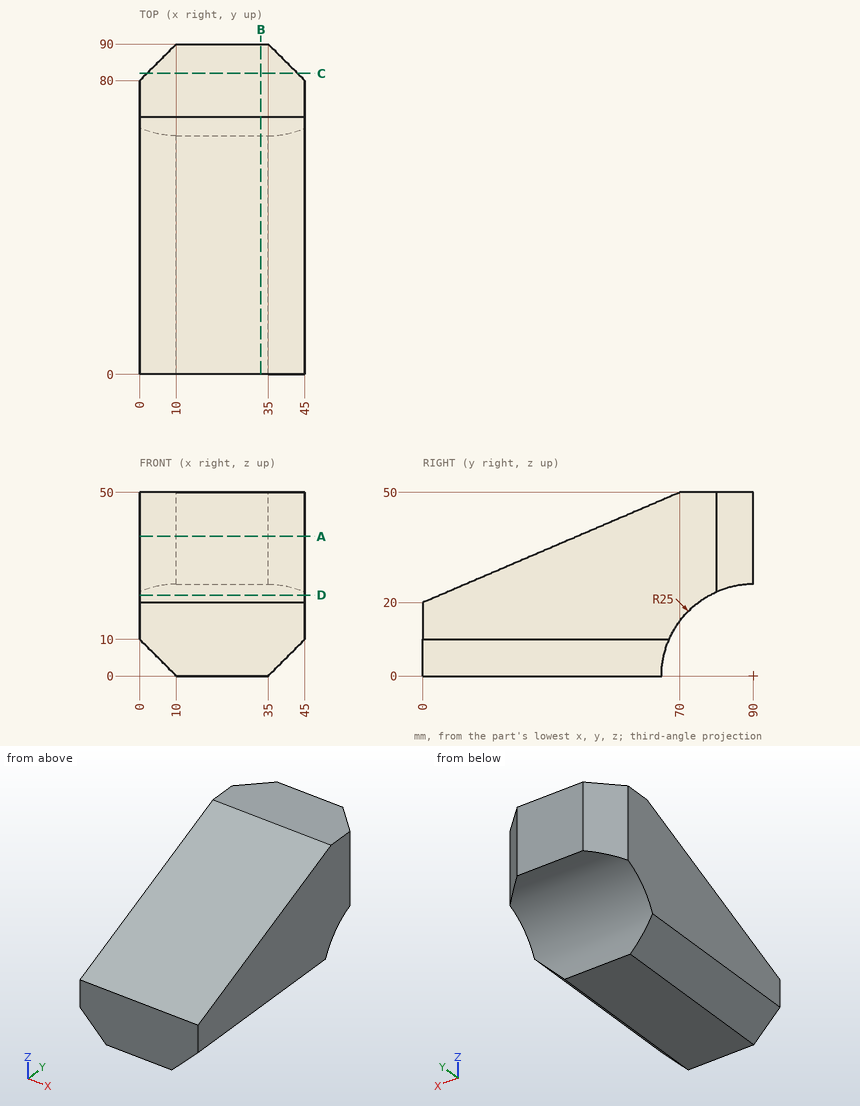
Geometry check sheet. Reference: drawing and pictorial views, mm from the part's lowest x, y, z. Give positions to 0.01 mm unless a question says otherwise; leave off trailing zeros. Loops run counter-clockwise (first coordinate to the right, second up) from the corner with the lowest first, then second, coordinate; pieces in that order, holes last.
1. Section check C-C, the plane y = 82. Enter the section's corners in (x, z), then the cut area to 3 significant figures.
2. Section check D-D, the plane z = 22. Enter the section's corners in (x, y), then the cut area to 3 significant figures.
3. Section check A-A, the plane z = 38. Enter the section's corners in (x, y).
4. Thickness scan on line 1 (Z direction, x = 35, y = 80); line 2 (Z direction, x = 27, y = 54); line 3 (Y direction, x = 25, z = 41.5). Record the ranges inside material, lowest first.
5. Go/stop test with flat-tipped pins: pin 1 Ø12 at (x, z) = (8.5, 33.5) entering from +Y; pin 2 Ø3 at (x, z) = (31, 8.5) entering from +Y; pin 3 Ø5 at (x, z) = (40, 27.5) entering from +Y; pin 4 Ø8 at (x, y) = (21.5, 29) entering from +Z. Record where each tip stops, or that it passes through.
6. Section check B-B, the plane x = 33. Enter the section's corners in (y, z), then the cut area to 3 significant figures.
Geometry says:
1. outline: (2, 23.69) - (43, 23.69) - (43, 50) - (2, 50) - close
1. area: 1,080 mm2
2. outline: (0, 4.67) - (45, 4.67) - (45, 78.13) - (0, 78.13) - close
2. area: 3,310 mm2
3. outline: (0, 42) - (45, 42) - (45, 80) - (35, 90) - (10, 90) - (0, 80) - close
4. line 1: z = 22.91 to 50
4. line 2: z = 0 to 43.14
4. line 3: y = 50.17 to 90
5. pin 1: stops at y = 90
5. pin 2: stops at y = 67.09
5. pin 3: stops at y = 87.5
5. pin 4: stops at z = 34.14
6. outline: (0, 0) - (65, 0) arc R25 cw to (90, 25) - (90, 50) - (70, 50) - (0, 20) - close
6. area: 2,960 mm2
